from build123d import *

# Parameters (mm, degrees)
SKETCH1_R           = 2
BOSS_EXTRUDE1_DEPTH = 5
SKETCH2_R           = 1
BOSS_EXTRUDE2_DEPTH = 4
BOSS_EXTRUDE3_DEPTH = 2
CHAMFER1_SIZE       = 0.5


with BuildPart() as part:
    # Sketch1 → Boss-Extrude1 (new body)
    with BuildSketch(Plane.XY):
        Circle(SKETCH1_R)
    extrude(amount=BOSS_EXTRUDE1_DEPTH)

    # Sketch2 → Boss-Extrude2 (add)
    with BuildSketch(Plane(origin=(0, 0, 0), x_dir=(-1, 0, 0), z_dir=(0, 0, -1))):
        Circle(SKETCH2_R)
    extrude(amount=BOSS_EXTRUDE2_DEPTH)

    # Sketch3 → Boss-Extrude3 (add)
    with BuildSketch(Plane(origin=(0, 0, -4), x_dir=(-1, 0, 0), z_dir=(0, 0, -1))):
        Polygon((0, 2.886751346), (-2.5, 1.443375673), (-2.5, -1.443375673), (0, -2.886751346), (2.5, -1.443375673), (2.5, 1.443375673), align=None)
    extrude(amount=BOSS_EXTRUDE3_DEPTH)

    # Chamfer1
    chamfer1_edges = [part.edges().sort_by_distance(p)[0] for p in [
        (-2, 0, 5),
    ]]
    chamfer(chamfer1_edges, length=CHAMFER1_SIZE)


solid = part.part
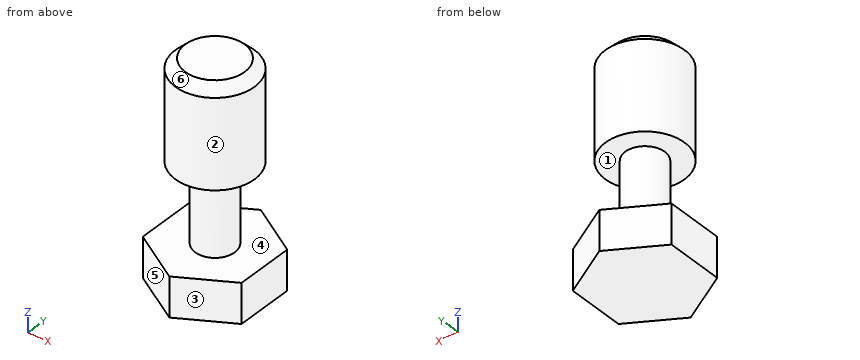
Verification items for the finished model (mm, model axes). Face numbers are marked on the shaded views. A direction names the side the tool comes from. Round coordinates to 2 decimals unless told otherwise and drop trailing zeros. Order: outer loops, then holes, each group sorted by start corner. A loop starts at its lowest first (then second) coordinate and runs counter-clockwise, first axis right, second up.
1. Access from +Z, -Z, +X, -X, +Y, -Y to the whole of each face (thin tool, end or side, straight path). Record for the marked faces 1, 2 and 3.
Final values:
face 1: none
face 2: +Z
face 3: +Z, -Z, +X, -Y
2. Release check for a two-part mould opening along Z. For the marked faces 4, 5 and 6 record: +Z half, -Z half, draft (parallel to the pull), parting line (faces both ways), or undercut.
Final values:
face 4: undercut
face 5: draft
face 6: +Z half
3. Section check D-D on z = 0.75. Record the cut outline in (x, y).
Final values:
outline: circle Ø4 at (0, 0)
4. Section check A-A on y = 0. Record the cut outline in (x, z).
Final values:
outline: (-2.5, -6) - (2.5, -6) - (2.5, -4) - (1, -4) - (1, 0) - (2, 0) - (2, 4.5) - (1.5, 5) - (-1.5, 5) - (-2, 4.5) - (-2, 0) - (-1, 0) - (-1, -4) - (-2.5, -4) - close
5. Section check C-C on y = -2.3. Record the cut outline in (x, z).
Final values:
outline: (-1.02, -6) - (1.02, -6) - (1.02, -4) - (-1.02, -4) - close
6. Section check B-B on z = -3.5. Record the cut outline in (x, y).
Final values:
outline: circle Ø2 at (0, 0)
7. Thickness scan on L1, parallel to Z at x = -0.9, y = 1.15; L2, parallel to Y at x = 0.1, z = 0.25; L3, parallel to Z at x = -0.1, y = 2.3. Record the ranges inside material, lowest first.
Final values:
L1: z = -6 to -4, 0 to 5
L2: y = -2 to 2
L3: z = -6 to -4
